Verification items for the finished model (mm, model axes). Face numbers are marked on the shaded views. Coordinates: 2 decimals unless noted, no trailing zeros. Order: outer loops, then holes, each group sorted by start corner. A loop starts at its lowest first (then second) coordinate and runs counter-clockwise, first axis right, second up. Notation, with made-up numbers: (21.25, 25) - (47.25, 25) arc R5 ccw to (47.25, 30) - close; hole circle Ø3 at (35, 58.5). An arc over 180 degrees is marked (long way). One line per question, with ' | ' between items. Start each with the question number.
from build123d import *

# Parameters (mm, degrees)
SKETCH_1_W          = 69
SKETCH_1_H          = 28
EXTRUDE_1_DEPTH     = 14
CUT_EXTRUDE_1_DEPTH = 47.585942086
CUT_EXTRUDE_2_DEPTH = 47.585942086


with BuildPart() as part:
    # 草图1 → 凸台-拉伸1 (new, symmetric)
    with BuildSketch(Plane.XY):
        Rectangle(SKETCH_1_W, SKETCH_1_H)
    extrude(amount=EXTRUDE_1_DEPTH, both=True)

    # 草图2 → 切除-拉伸1 (cut, through all)
    with BuildSketch(Plane.XY.offset(14)):
        with BuildLine():
            Line((-34.5, 1), (-22.449874371, 1))
            ThreePointArc((-22.449874371, 1), (-2.5, 0), (-22.449874371, -1))
            Line((-22.449874371, -1), (-34.5, -1))
            Line((-34.5, -1), (-34.5, 1))
        make_face()
    extrude(amount=-CUT_EXTRUDE_1_DEPTH, mode=Mode.SUBTRACT)

    # 草图3 → 切除-拉伸2 (cut, through all)
    with BuildSketch(Plane(origin=(0, 14, 0), x_dir=(1, 0, 0), z_dir=(0, 1, 0))):
        with BuildLine():
            Line((22.449874371, -1), (34.5, -1))
            Line((34.5, -1), (34.5, 1))
            Line((34.5, 1), (22.449874371, 1))
            ThreePointArc((22.449874371, 1), (2.5, 0), (22.449874371, -1))
        make_face()
    extrude(amount=-CUT_EXTRUDE_2_DEPTH, mode=Mode.SUBTRACT)


solid = part.part
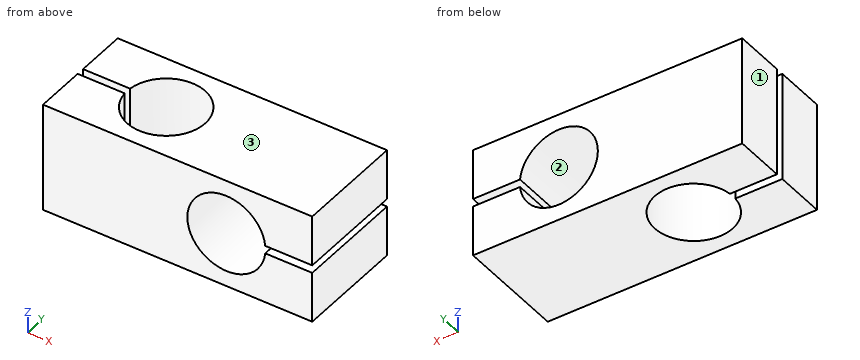
Item 1: Section check C-C (z = 0). Record the cut outline in (x, y).
Item 2: Thickness scan on probe 1 along Y at (x, z) = (-12.5, 7.5); probe 2 along Z at (x, y) = (13, 12.5); probe 3 along X at (y, z) = (-5.5, -8). Record the ranges inside material, lowest first. Write a range as from..to.
Item 3: Section check B-B (y = -1.75). Record the cut outline in (x, z).
Item 4: Section check A-A (x = -12.5). Record the cut outline in (y, z), then the cut area to 3 significant figures.
Item 5: Section check D-D (z = -8.5). Record the cut outline in (x, y).
Item 6: Mould release check, pull along Z, two halves, no side actions. Record for the marked faces 1, 2 and 3: +Z half, -Z half, draft (parallel to the pull), parting line (faces both ways), or undercut.
Completed:
1) outline: (-34.5, -14) - (2.5, -14) - (2.5, 14) - (-34.5, 14) - (-34.5, 1) - (-22.45, 1) arc R10 cw (long way) to (-22.45, -1) - (-34.5, -1) - close
2) probe 1: y = -14..-10, 10..14 | probe 2: z = -14..-9.99, 9.99..14 | probe 3: x = -34.5..-20.85, -4.15..6.5, 18.5..34.5
3) outline: (-34.5, -14) - (-22.35, -14) - (-22.35, 14) - (-34.5, 14) - close; (-2.65, -14) - (34.5, -14) - (34.5, -1) - (22.45, -1) arc R10 cw (long way) to (22.45, 1) - (34.5, 1) - (34.5, 14) - (-2.65, 14) - close
4) outline: (-14, -14) - (-10, -14) - (-10, 14) - (-14, 14) - close; (10, -14) - (14, -14) - (14, 14) - (10, 14) - close | area: 224 mm^2
5) outline: (-34.5, -14) - (7.23, -14) - (7.23, 14) - (-34.5, 14) - (-34.5, 1) - (-22.45, 1) arc R10 cw (long way) to (-22.45, -1) - (-34.5, -1) - close; (17.77, -14) - (34.5, -14) - (34.5, 14) - (17.77, 14) - close
6) face 1: draft | face 2: undercut | face 3: +Z half
